Part model, mm, in its own coordinate system. A direction names the side the tool comes from. Give positions to 0.01 mm unless a question says otherwise; leave off trailing zeros. Order: outer loops, then holes, each group sorted by start corner. A loop starts at its lowest first (then second) coordinate and runs counter-clockwise, first axis right, second up. Notation, with made-up numbers: M 59,-9.5 L 111,-9.5 A11 ccw 111,-1.5 Z; hole C -4,88 d6. An arc over 180 degrees is marked long. Answer as a JSON object with one key per item and string values.
from build123d import *

# Parameters (mm, degrees)
SKETCH_1_R      = 6
EXTRUDE_1_DEPTH = 10


with BuildPart() as part:
    # 草图1 → 凸台-拉伸1 (new body)
    with BuildSketch(Plane.XY):
        with BuildLine():
            Line((0, 0), (130, 0))
            Line((130, 0), (130, 190))
            Line((130, 190), (105, 190))
            Line((105, 190), (105, 150))
            ThreePointArc((105, 150), (65, 110), (25, 150))
            Line((25, 150), (25, 190))
            Line((25, 190), (0, 190))
            Line((0, 190), (0, 0))
        make_face()
        with Locations((117.5, 150)):
            Circle(SKETCH_1_R, mode=Mode.SUBTRACT)
        with Locations((12.5, 150)):
            Circle(SKETCH_1_R, mode=Mode.SUBTRACT)
        with Locations((40, 25)):
            Circle(SKETCH_1_R, mode=Mode.SUBTRACT)
        with Locations((90, 25)):
            Circle(SKETCH_1_R, mode=Mode.SUBTRACT)
    extrude(amount=EXTRUDE_1_DEPTH)


solid = part.part
1. Two-plate mould, pull along X, no slides. Class faces 1 (the flat face through (130, 94, 5)), 2 (the flat face through (13, 190, 5)), 3 (the cylindrical face through (84, 25, 5)): +X half, -X half, draft (parallel to the pull), parting line (faces both ways), or undercut.
Worked answers:
{"face 1": "+X half", "face 2": "draft", "face 3": "undercut"}
2. Pin check, flat tip, straight feed: P1, Ø14, axis at x = 12.5, y = 150, coming from the -Z side. Stop position of the tip, or through.
Worked answers:
{"P1": "stops at z = 0"}
3. Cut at D-D on z = 7.75. Give the cut face in (x, y), plus the area to 3 significant figures.
Worked answers:
{"outline": "M 0,0 L 130,0 L 130,190 L 105,190 L 105,150 A40 cw 25,150 L 25,190 L 0,190 Z; hole C 12.5,150 d12; hole C 40,25 d12; hole C 90,25 d12; hole C 117.5,150 d12", "area": "18,500 mm^2"}
4. Probe line 1 along X through (y, z) = (146, 0.5); line 2 along X through (y, z) = (181, 6.75); line 3 along Y through (x, z) = (15, 4.75). List the from-to ranges inside material, lowest first.
Worked answers:
{"line 1": "x = 0 to 8.03, 16.97 to 25.2, 104.8 to 113.03, 121.97 to 130", "line 2": "x = 0 to 25, 105 to 130", "line 3": "y = 0 to 144.55, 155.45 to 190"}
5. Which spindle directions (+Z, -Z, +X, -X, +Y, -Y) get a long thin tool onto all of the face, cutting with end or side? Do faces 4 (the flat face through (64, 75, 0)), 5 (the flat face through (25, 170, 5)). Say none if no direction does.
Worked answers:
{"face 4": "-Z, +X, -X, +Y, -Y", "face 5": "+Z, -Z, +Y"}
6. Cut at B-B on x = 117.5. Give the cut face in (y, z).
Worked answers:
{"outline": "M 0,0 L 144,0 L 144,10 L 0,10 Z; M 156,0 L 190,0 L 190,10 L 156,10 Z"}
7. Cut at A-A on y = 25. Give the cut face in (x, z), plus the area to 3 significant figures.
Worked answers:
{"outline": "M 0,0 L 34,0 L 34,10 L 0,10 Z; M 46,0 L 84,0 L 84,10 L 46,10 Z; M 96,0 L 130,0 L 130,10 L 96,10 Z", "area": "1,060 mm^2"}
8. Cut at C-C on y = 166.5. Give the cut face in (x, z).
Worked answers:
{"outline": "M 0,0 L 25,0 L 25,10 L 0,10 Z; M 105,0 L 130,0 L 130,10 L 105,10 Z"}
